Input: part model. Units: mm. Frame: model coordinates. A direction names the side the tool comes from. Give positions to 0.01 mm unless a question says otherwise; leave off trailing zeros. Loops run counter-clockwise (first coordinate to the right, second up) from the corner with the lowest first, then second, coordinate; pieces in that order, holes last. Notation, with made-up numbers: M 77,-4.75 L 96,-4.75 A17 cw 96,22.25 Z; hole C 64,-4 d4. An arc over 180 degrees is marked long. One line per item, written item: value. Start each with the question number.
(1) Ray query, line 1 along X through (y, z) = (6, -8.5); line 2 along X through (y, z) = (-10.5, -2); line 3 along Z through (x, y) = (48, -4.5). Return the intervals inside material, ascending. Write a range as from..to.
(2) Access query for faces 1 (the conical face through (0.224, -5.421, -9.442)), 2 (the flat face through (8.8, -9, 0)). Directions: +Z, -Z, +X, -X, +Y, -Y. A direction counts if a zero-diameter tool reaches every point of the face in a straight line with its end or side. Return the directions, or none.
(3) Section A-A on x = 6. Output: boundary loops of the cut face in (y, z).
(4) Section B-B on x = 56.5. Output: boundary loops of the cut face in (y, z), plus the area to 3 significant figures.
(5) Pin query (flat end, axial travel): P1, Ø1, axis at x = 39.5, z = 5.5, coming from the +Y side; P2, Ø12, axis at x = 49.5, z = -2.5, coming from the -Y side; P3, Ø1, axis at y = 4.5, z = -8, coming from the +X side. Return the tip coordinate at first contact, or that it passes through.
```python
from build123d import *

# Parameters (mm, degrees)
BOSS_EXTRUDE1_DEPTH = 8.8
SKETCH4_R           = 22.78
SKETCH4_R_2         = 10.5
CUT_EXTRUDE1_DEPTH  = 1.1
CUT_EXTRUDE1_DRAFT  = -60
CHAMFER2_SIZE       = 0.777777778


with BuildPart() as part:
    # Sketch3 → Boss-Extrude1 (new body)
    with BuildSketch(Plane(origin=(0, 0, 0), x_dir=(0, 0, -1), z_dir=(1, 0, 0))):
        Polygon((10.5, 6.062177826), (0, 12.124355653), (-10.5, 6.062177826), (-10.5, -6.062177826), (0, -12.124355653), (10.5, -6.062177826), align=None)
    extrude(amount=BOSS_EXTRUDE1_DEPTH)


with BuildPart() as cut_extrude1_tool:
    # Sketch4 → Cut-Extrude1 (with draft: the straight prism first)
    with BuildSketch(Plane.ZY):
        Circle(SKETCH4_R)
        Circle(SKETCH4_R_2, mode=Mode.SUBTRACT)
    extrude(amount=-CUT_EXTRUDE1_DEPTH)
    # Cut-Extrude1: the draft: its side faces are tilted about the plane it starts from
    cut_extrude1_sides = [cut_extrude1_tool.faces().sort_by_distance(p)[0] for p in [
        (0.55, 0, -22.78),
        (0.55, 0, -10.5),
    ]]
    draft(cut_extrude1_sides, Plane.ZY, CUT_EXTRUDE1_DRAFT)


with BuildPart() as part_1:
    add(part.part)

    # Cut-Extrude1: cut by cut_extrude1_tool
    add(cut_extrude1_tool.part, mode=Mode.SUBTRACT)

    # Sketch5 → Revolve1 (revolve)
    with BuildSketch(Plane.XY, mode=Mode.PRIVATE) as revolve1_sk:
        with BuildLine():
            Line((10.15, 7), (73.8, 7))
            Line((73.8, 7), (73.8, 0))
            Line((73.8, 0), (8.8, 0))
            Line((8.8, 0), (8.8, 8.35))
            ThreePointArc((8.8, 8.35), (9.195405845, 7.395405845), (10.15, 7))
        make_face()
    revolve(revolve1_sk.sketch.rotate(Axis((8.8, 0, 0), (1, 0, 0)), 90), axis=Axis((8.8, 0, 0), (1, 0, 0)))

    # Chamfer2
    chamfer2_edges = [part_1.edges().sort_by_distance(p)[0] for p in [
        (73.8, 0, -7),
    ]]
    chamfer(chamfer2_edges, length=CHAMFER2_SIZE)


solid = part_1.part
```
Output values:
1. line 1: x = 0..8.8
1. line 2: x = 0.11..8.8
1. line 3: z = -5.36..5.36
2. face 1: -Z, -X, -Y
2. face 2: +X
3. outline: M -12.12,0 L -6.06,-10.5 L 6.06,-10.5 L 12.12,0 L 6.06,10.5 L -6.06,10.5 Z
4. outline: C 0,0 d14
4. area: 154 mm²
5. P1: stops at y = 4.9
5. P2: stops at y = -7
5. P3: stops at x = 8.8
